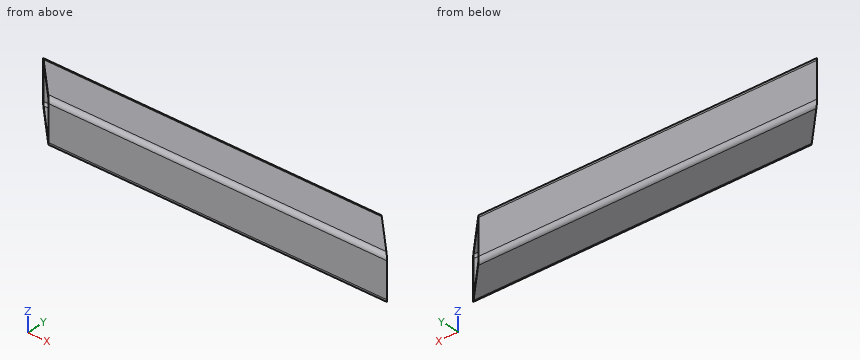
from build123d import *

# Parameters (mm, degrees)
F_100_X_100_X_5_1_DEPTH = 900
CUT_EXTRUDE_1_DEPTH     = 100


with BuildPart() as part:
    # Sketch1 → 方形管 100 X 100 X 5(1) (new body)
    with BuildSketch(Plane(origin=(0, 0, 0), x_dir=(0, 0, -1), z_dir=(1, 0, 0))):
        with BuildLine():
            Line((-40, -50), (40, -50))
            ThreePointArc((40, -50), (47.071067812, -47.071067812), (50, -40))
            Line((50, -40), (50, 40))
            ThreePointArc((50, 40), (47.071067812, 47.071067812), (40, 50))
            Line((40, 50), (-40, 50))
            ThreePointArc((-40, 50), (-47.071067812, 47.071067812), (-50, 40))
            Line((-50, 40), (-50, -40))
            ThreePointArc((-50, -40), (-47.071067812, -47.071067812), (-40, -50))
        make_face()
        with BuildLine():
            Line((-40, -45), (40, -45))
            ThreePointArc((40, -45), (43.535533906, -43.535533906), (45, -40))
            Line((45, -40), (45, 40))
            ThreePointArc((45, 40), (43.535533906, 43.535533906), (40, 45))
            Line((40, 45), (-40, 45))
            ThreePointArc((-40, 45), (-43.535533906, 43.535533906), (-45, 40))
            Line((-45, 40), (-45, -40))
            ThreePointArc((-45, -40), (-43.535533906, -43.535533906), (-40, -45))
        make_face(mode=Mode.SUBTRACT)
    extrude(amount=F_100_X_100_X_5_1_DEPTH)

    # 草图2 → 切除-拉伸1 (cut)
    with BuildSketch(Plane.XY.offset(50)):
        Polygon((0, 50), (100, -50), (0, -50), align=None)
        Polygon((913.789188304, -85.971728999), (913.789188304, 50), (777.817459305, 50), align=None)
    extrude(amount=-CUT_EXTRUDE_1_DEPTH, mode=Mode.SUBTRACT)


solid = part.part
Design review of the part built by this model. Coordinates are the model's own, in mm. Coordinates: 2 decimals unless noted, no trailing zeros. Loops run counter-clockwise (first coordinate to the right, second up) from the corner with the lowest first, then second, coordinate; pieces in that order, holes last. Notation, with made-up numbers: M 25,11.25 L 30,11.25 A11 ccw 30,30.25 Z; hole C -34.75,66.25 d11. An arc over 180 degrees is marked long. Answer as CSV lines item,"result".
Item 1: Add section C-C on z = -15. State the section outline as (x, y) points, plus the area to 3 significant figures.
Answer list:
outline,"M 0,50 L 5,45 L 782.82,45 L 777.82,50 Z; M 95,-45 L 100,-50 L 877.82,-50 L 872.82,-45 Z"
area,"7,780 mm²"
Item 2: Add section A-A on x = 491. State the section outline as (y, z) points, plus the area to 3 significant figures.
Answer list:
outline,"M -50,-40 A10 ccw -40,-50 L 40,-50 A10 ccw 50,-40 L 50,40 A10 ccw 40,50 L -40,50 A10 ccw -50,40 Z; hole M -45,-40 A5 ccw -40,-45 L 40,-45 A5 ccw 45,-40 L 45,40 A5 ccw 40,45 L -40,45 A5 ccw -45,40 Z"
area,"1,840 mm²"
Item 3: For probe 1 along Z at (x, y) = (59, 20.5); probe 2 along Z at (x, y) = (771, 41), list the stretches that pass through material, from the lowest coordinate up.
Answer list:
probe 1,"-50 to -45, 45 to 50"
probe 2,"-49.95 to -44.9, 44.9 to 49.95"
Item 4: Add section D-D on x = 820. State the section outline as (y, z) points.
Answer list:
outline,"M -50,-40 A10 ccw -40,-50 L 7.82,-50 L 7.82,-45 L -40,-45 A5 cw -45,-40 L -45,40 A5 cw -40,45 L 7.82,45 L 7.82,50 L -40,50 A10 ccw -50,40 Z"
Item 5: Add section B-B on y = -16.5. State the section outline as (x, z) points, plus the area to 3 significant figures.
Answer list:
outline,"M 66.5,-50 L 844.32,-50 L 844.32,-45 L 66.5,-45 Z; M 66.5,45 L 844.32,45 L 844.32,50 L 66.5,50 Z"
area,"7,780 mm²"
